```python
from build123d import *

# Parameters (mm, degrees)
LINK_BODY_DEPTH        = 10
PIN_HOLES_SKETCH_R     = 4
PIN_HOLES_2X_8_DEPTH   = 10
SIDE_SLOTS_SKETCH_R    = 5
SIDE_SLOTS_SKETCH_W    = 30.75281097
SIDE_SLOTS_SKETCH_H    = 5
SIDE_SLOTS_SKETCH_W_2  = 29.537366276
SIDE_SLOTS_CUT_DEPTH   = 10
COUNTERBORE_SKETCH_R   = 9
COUNTERBORE_18X2_DEPTH = 2


with BuildPart() as part:
    # Link Body Sketch → Link Body (new, symmetric)
    with BuildSketch(Plane(origin=(0, 0, 0), x_dir=(1, 0, 0), z_dir=(0, 1, 0))):
        with BuildLine():
            Line((10, 30), (10, -30))
            ThreePointArc((10, -30), (0, -40), (-10, -30))
            Line((-10, -30), (-10, 30))
            ThreePointArc((-10, 30), (0, 40), (10, 30))
        make_face()
    extrude(amount=LINK_BODY_DEPTH, both=True)

    # Pin Holes Sketch → Pin Holes 2xØ8 (cut, symmetric)
    with BuildSketch(Plane(origin=(0, 0, 0), x_dir=(1, 0, 0), z_dir=(0, 1, 0))):
        with Locations(Location((0, 30, 0), (0, 0, 270))):
            Circle(PIN_HOLES_SKETCH_R)
        with Locations(Location((0, -30, 0), (0, 0, 270))):
            Circle(PIN_HOLES_SKETCH_R)
    extrude(amount=PIN_HOLES_2X_8_DEPTH, both=True, mode=Mode.SUBTRACT)

    # Side Slots Sketch → Side Slots Cut (cut, symmetric)
    with BuildSketch(Plane(origin=(0, 0, 0), x_dir=(0, 0, -1), z_dir=(1, 0, 0))):
        Circle(SIDE_SLOTS_SKETCH_R)
        with Locations((-30.376405485, 0)):
            Rectangle(SIDE_SLOTS_SKETCH_W, SIDE_SLOTS_SKETCH_H)
        with Locations((29.768683138, 0)):
            Rectangle(SIDE_SLOTS_SKETCH_W_2, SIDE_SLOTS_SKETCH_H)
    extrude(amount=SIDE_SLOTS_CUT_DEPTH, both=True, mode=Mode.SUBTRACT)

    # Counterbore Sketch → Counterbore Ø18x2 (cut)
    with BuildSketch(Plane(origin=(10, 0, 0), x_dir=(0, 0, -1), z_dir=(1, 0, 0))):
        Circle(COUNTERBORE_SKETCH_R)
    extrude(amount=-COUNTERBORE_18X2_DEPTH, mode=Mode.SUBTRACT)


solid = part.part
```
Could you check a few things on this model? Use its own coordinates, in mm. A direction names the side the tool comes from. Round coordinates to 2 decimals unless told otherwise and drop trailing zeros. Loops run counter-clockwise (first coordinate to the right, second up) from the corner with the lowest first, then second, coordinate; pieces in that order, holes last.
Q1. Please list where these lines run through material, in increasing order: L1, parallel to X at y = 5.5, z = -30; L2, parallel to Y at x = 6, z = -32.5; L3, parallel to Y at x = 8.9, z = 0.
Q2. I want a section at C-C (x = 0). Give the number of separate pieces and of enclosed holes in the cut face, and give its area (3 significant figures).
Q3. Thinking about a two-plate mould opening in Z: for faces 4 (the cylindrical face through (9.014, 8.923, 1.172)), 5 (the flat face through (0, -2.5, -25)), 6 (the cylindrical face through (0, -6, -40)), which applies, pulls with the +Z half, pulls with the -Z half, needs draft (parallel to the pull), parting line crosses it, or undercut?
Q4. I want a section at D-D (z = 0). Write out the boundary of the cut face in (x, y).
Q5. I want a section at B-B (y = 0). Write out the boundary of the cut face in (x, z), and give its area (3 significant figures).
Q6. For P1, Ø2.5, axis at x = 5, y = 0, coming from the +Z side; P2, Ø1.5, axis at x = 3.5, y = 3.5, coming from the +Z side; P3, Ø9, axis at y = 2.5, z = 1, coming from the +X side, each with a flat end and sliding along its axis, tell me the tip position at first contact or that it passes through.
Q7. I want a section at A-A (z = 25). Write out the boundary of the cut face in (x, y).
Q8. On a 3-axis mill with a long thin cutter (end or side, diameter ignored), from which of +Z, -Z, +X, -X, +Y, -Y can I reach the whole of each face in a straight line? I mean faces 1 (the flat face through (0, 0, -15)), 2 (the flat face through (0, 0, 15)), 3 (the flat face through (8, -4, -4)). Say none if no direction works.
Answer below:
1. L1: x = -10 to -4, 4 to 10
1. L2: y = -10 to -2.5, 2.5 to 10
1. L3: y = -10 to -9, 9 to 10
2. separate pieces: 5
2. enclosed holes: 1
2. area: 1,030 mm2
3. face 4: undercut
3. face 5: needs draft
3. face 6: pulls with the -Z half
4. outline: (-10, -10) - (10, -10) - (10, -9) - (8, -9) - (8, -5) - (-10, -5) - close; (-10, 5) - (8, 5) - (8, 9) - (10, 9) - (10, 10) - (-10, 10) - close
5. outline: (-10, -15) - (10, -15) - (10, -9) - (8, -9) - (8, -5) - (-10, -5) - close; (-10, 5) - (8, 5) - (8, 9) - (10, 9) - (10, 15) - (-10, 15) - close
5. area: 384 mm2
6. P1: stops at z = 15
6. P2: stops at z = 39.61
6. P3: stops at x = 8
7. outline: (-10, -10) - (10, -10) - (10, -2.5) - (-10, -2.5) - close; (-10, 2.5) - (10, 2.5) - (10, 10) - (-10, 10) - close
8. face 1: -Z, +X, -X
8. face 2: +Z, +X, -X
8. face 3: +X
